from build123d import *

# Parameters (mm, degrees)
CUT_EXTRUDE_1_DEPTH      = 101.279609094
CUT_EXTRUDE_1_DEPTH_BACK = 101.279609094
SKETCH_2_R               = 8.75


with BuildPart() as part:
    # 草图1 → 旋转1 (revolve)
    with BuildSketch(Plane(origin=(0, 0, 0), x_dir=(1, 0, 0), z_dir=(0, 1, 0)), mode=Mode.PRIVATE) as revolve_1_sk:
        Polygon((0, 21.5), (0, 70), (16, 70), (16, 41), (18, 39), (18, 21.5), align=None)
    revolve(revolve_1_sk.sketch.rotate(Axis((0, 0, 0), (1, 0, 0)), 180), axis=Axis((0, 0, 0), (1, 0, 0)))

    # 草图2 → 切除-拉伸1 (cut, two sides: drawn at the far end of the back side and taken through both)
    with BuildSketch(Plane(origin=(16, 0, 0), x_dir=(0, 0, -1), z_dir=(1, 0, 0)).offset(-CUT_EXTRUDE_1_DEPTH_BACK)):
        with Locations((0, 50)):
            Circle(SKETCH_2_R)
        with Locations((50, 0)):
            Circle(SKETCH_2_R)
        with Locations((0, -50)):
            Circle(SKETCH_2_R)
        with Locations((-50, 0)):
            Circle(SKETCH_2_R)
    extrude(amount=CUT_EXTRUDE_1_DEPTH + CUT_EXTRUDE_1_DEPTH_BACK, mode=Mode.SUBTRACT)


solid = part.part
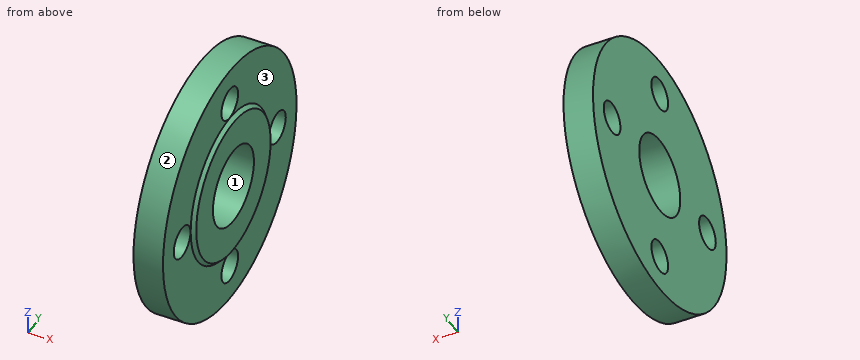
For this review, take the finished solid that the model builds, in its own axes (mm). Face numbers are marked on the shaded views. Round coordinates to 2 decimals unless told otherwise and drop trailing zeros. Loops run counter-clockwise (first coordinate to the right, second up) from the corner with the lowest first, then second, coordinate; pieces in that order, holes last. Notation, with made-up numbers: (32.25, 0.25) - (46.25, 0.25) arc R15 ccw to (46.25, 10.25) - close; hole circle Ø4 at (65.5, 76.25). An arc over 180 degrees is marked (long way). Put each result on its own line as item: value. Start each with the question number.
1. Consider section D-D on z = -50. State the section outline as (x, y) points.
2. Insertion check: P1, Ø16, axis at y = 0, z = 50, coming from the -X side; P2, Ø4, axis at x = 2, z = 10.5, coming from the +Y side; P3, Ø1.5, axis at x = 7, z = -25.5, coming from the +Y side; P4, Ø20, axis at y = -50, z = 0, coming from the +X side. Each pin has a flat end and moves straight along its axis. Give the tip position at first contact, or say it passes through.
3. Consider section B-B on y = -46. State the section outline as (x, z) points.
4. Mouldability with a two-part tool opening along Z and no side actions: class the marked faces 1, 2 and 3 as +Z half, -Z half, draft (parallel to the pull), parting line (faces both ways), or undercut.
5. Consider section C-C on x = 12.5. State the section outline as (y, z) points.
6. For probe 1 along Y at (x, z) = (9, 0); probe 2 along Y at (x, z) = (5, 56); probe 3 along Z at (x, y) = (11.25, -43), list the stretches that pass through material, from the lowest coordinate up. Write a range as [from, to].
7. Consider section A-A on z = 0. State the section outline as (x, y) points.
Result sheet:
1. outline: (0, -48.99) - (16, -48.99) - (16, -8.75) - (0, -8.75) - close; (0, 8.75) - (16, 8.75) - (16, 48.99) - (0, 48.99) - close
2. P1: through
2. P2: y = 69.48
2. P3: y = 65.48
2. P4: x = 17
3. outline: (0, -52.76) - (16, -52.76) - (16, -7.78) - (0, -7.78) - close; (0, 7.78) - (16, 7.78) - (16, 52.76) - (0, 52.76) - close
4. face 1: undercut
4. face 2: parting line
4. face 3: draft
5. outline: circle Ø140 at (0, 0); hole circle Ø17.5 at (-50, 0); hole circle Ø43 at (0, 0); hole circle Ø17.5 at (0, -50); hole circle Ø17.5 at (0, 50); hole circle Ø17.5 at (50, 0)
6. probe 1: [-70, -58.75], [-41.25, -21.5], [21.5, 41.25], [58.75, 70]
6. probe 2: [-42, -6.37], [6.37, 42]
6. probe 3: [-55.24, -5.25], [5.25, 55.24]
7. outline: (0, -70) - (16, -70) - (16, -58.75) - (0, -58.75) - close; (0, -41.25) - (16, -41.25) - (16, -41) - (18, -39) - (18, -21.5) - (0, -21.5) - close; (0, 21.5) - (18, 21.5) - (18, 39) - (16, 41) - (16, 41.25) - (0, 41.25) - close; (0, 58.75) - (16, 58.75) - (16, 70) - (0, 70) - close
